```python
from build123d import *

# Parameters (mm, degrees)
SKETCH4_R          = 90
CUT_EXTRUDE1_DEPTH = 343
CIRPATTERN1_COUNT  = 6
CIRPATTERN2_COUNT  = 3
SKETCH8_R          = 12.5
CUT_EXTRUDE3_DEPTH = 238


with BuildPart() as part:
    # Sketch2 → Revolve1 (revolve)
    with BuildSketch(Plane.XY, mode=Mode.PRIVATE) as revolve1_sk:
        with BuildLine():
            Line((-20, 600), (-20, 530))
            Line((-20, 530), (80, 530))
            ThreePointArc((80, 530), (90.606601718, 525.606601718), (95, 515))
            Line((95, 515), (95, 205))
            ThreePointArc((95, 205), (87.67766953, 187.32233047), (70, 180))
            Line((70, 180), (0, 180))
            Line((0, 180), (0, 105))
            Line((0, 105), (70, 105))
            Line((70, 105), (70, 80))
            Line((70, 80), (240, 80))
            Line((240, 80), (240, 150))
            Line((240, 150), (170, 150))
            ThreePointArc((170, 150), (152.32233047, 157.32233047), (145, 175))
            Line((145, 175), (145, 515))
            ThreePointArc((145, 515), (149.393398282, 525.606601718), (160, 530))
            Line((160, 530), (260, 530))
            Line((260, 530), (260, 600))
            Line((260, 600), (-20, 600))
        make_face()
    revolve(revolve1_sk.sketch.rotate(Axis((225.657059372, 0, 0), (-1, 0, 0)), 90), axis=Axis((225.657059372, 0, 0), (-1, 0, 0)))

    # Sketch4 → Cut-Extrude1 (cut)
    with BuildSketch(Plane(origin=(0, 0, 0), x_dir=(0, 0, -1), z_dir=(1, 0, 0))):
        with Locations(Location((-170, 294.448637287, 0), (0, 0, 180))):
            Circle(SKETCH4_R)
    cut_extrude1 = extrude(amount=CUT_EXTRUDE1_DEPTH, mode=Mode.SUBTRACT)

    # CirPattern1: Cut-Extrude1 ×6 about axis
    cirpattern1_axis = Axis((0, 0, 0), (1, 0, 0))
    for i in range(1, CIRPATTERN1_COUNT):
        add(cut_extrude1.rotate(cirpattern1_axis, i * 360 / CIRPATTERN1_COUNT), mode=Mode.SUBTRACT)

    # Sketch6 → M24 Tapped Hole1 (revolve, cut)
    with BuildSketch(Plane(origin=(0, 114.748366001, 66.25), x_dir=(0, 0, 1), z_dir=(0, 1, 0))):
        Polygon((0, 0), (0, 46.3090365), (10.5, 40), (10.5, 0), align=None)
    m24_tapped_hole1 = revolve(axis=Axis((-6.35, 114.748366001, 66.25), (1, 0, 0)), mode=Mode.SUBTRACT)

    # CirPattern2: M24 Tapped Hole1 ×3 about axis
    cirpattern2_axis = Axis((0, 0, 0), (1, 0, 0))
    for i in range(1, CIRPATTERN2_COUNT):
        add(m24_tapped_hole1.rotate(cirpattern2_axis, i * 360 / CIRPATTERN2_COUNT), mode=Mode.SUBTRACT)

    # Sketch8 → Cut-Extrude3 (cut)
    with BuildSketch(Plane(origin=(0, 0, 0), x_dir=(0, 0, -1), z_dir=(1, 0, 0))):
        with Locations(Location((-55, -462, 0), (0, 0, 180))):
            Circle(SKETCH8_R)
        with Locations(Location((-165, -462, 0), (0, 0, 180))):
            Circle(SKETCH8_R)
        with Locations(Location((55, -462, 0), (0, 0, 180))):
            Circle(SKETCH8_R)
        with Locations(Location((165, -462, 0), (0, 0, 180))):
            Circle(SKETCH8_R)
    extrude(amount=CUT_EXTRUDE3_DEPTH, mode=Mode.SUBTRACT)


solid = part.part
```
Part model, mm, in its own coordinate system. A direction names the side the tool comes from. Round coordinates to 2 decimals unless told otherwise and drop trailing zeros. Order: outer loops, then holes, each group sorted by start corner. A loop starts at its lowest first (then second) coordinate and runs counter-clockwise, first axis right, second up. Notation, with made-up numbers: M -35.75,44 L -7.75,44 A32 cw -7.75,79 Z; hole C -20.75,80.25 d10. An arc over 180 degrees is marked long. Answer in a Markdown table with one row per item. Add a question column.
Q1. Cut at B-B on y = -318. Give the number of separate pieces and of enclosed holes in the cut face, and give its area (3 significant figures).
Q2. Wall check: L1, parallel to Y at x = 196, z = 0; L2, parallel to Y at x = 166, z = 68.5; L3, parallel to Z at x = 119, y = -333. Give the ranges that are in metal, low to high. Write a range as from..to.
Q3. Cut at A-A on x = 206.5. Give the cut face in (y, z), and give its area (3 significant figures).
Q4. 3-axis set-ups, long thin cutter, end or side, ignore diameter. For faces 1 (the face through (95, 222, 7)), 2 (the face through (119.65, -34.471, 256.863)), 3 (the face through (240, 65, 65)): which of +Z, -Z, +X, -X, +Y, -Y reach the whole face in a straight line?
Q5. Pin check, flat tips, straight feed: pin 1 (8 mm diameter, centred on x = 112, y = -357, fed in from -Z); pin 2 (3 mm diameter, centred on x = 43, y = -420.5, fed in from -Z); pin 3 (3 mm diameter, centred on x = 150.5, y = 37, fed in from +Z). Stop position of each tip, or through.
Q6. Mould opens along Z. For faces 4 (the face through (118.04, 532.303, -276.863)), 5 (the face through (119.65, -370.34, 218.38)), 6 (the face through (-20, 531, 3)) say: +Z half, -Z half, draft (parallel to the pull), parting line (faces both ways), or undercut.
Established:
| question | item | result |
|---|---|---|
| 1 | separate pieces | 3 |
| 1 | enclosed holes | 0 |
| 1 | area | 72,800 mm2 |
| 2 | L1 | y = -600..-530, -150..-80, 80..150, 530..600 |
| 2 | L2 | y = -596.08..-525.55, -133.81..-41.32, 41.32..133.81, 525.55..596.08 |
| 2 | L3 | z = -499.11..-251.33, -88.67..88.67, 251.33..499.11 |
| 3 | outline | C 0,0 d1200; C 0,0 d300; hole C 0,0 d1060; hole C 0,0 d160 |
| 3 | area | 299,000 mm2 |
| 4 | face 1 | -X |
| 4 | face 2 | +X, -X |
| 4 | face 3 | +X |
| 5 | pin 1 | stops at z = -485.17 |
| 5 | pin 2 | stops at z = -429.46 |
| 5 | pin 3 | stops at z = 598.95 |
| 6 | face 4 | parting line |
| 6 | face 5 | undercut |
| 6 | face 6 | draft |
